Can you work these out from the model? Positions are in its coordinate system, mm. A direction names the side the tool comes from. Give positions to 0.01 mm unless a question says otherwise; leave off trailing zeros. Loops run counter-clockwise (first coordinate to the right, second up) from the corner with the lowest first, then second, coordinate; pieces in that order, holes last. Notation, with made-up numbers: (53.5, -12.5) - (95.5, -12.5) arc R23 ccw to (95.5, -4.5) - close; hole circle Ø6 at (4.25, 79). An arc over 180 degrees is marked (long way). Write item = value, one per line.
from build123d import *

# Parameters (mm, degrees)
SKETCH1_W           = 70
SKETCH1_H           = 100
BOSS_EXTRUDE1_DEPTH = 30
SKETCH2_R           = 4
BOSS_EXTRUDE2_DEPTH = 4
SKETCH3_W           = 35
SKETCH3_H           = 100
BOSS_EXTRUDE3_DEPTH = 40
SKETCH4_R           = 10
BOSS_EXTRUDE4_DEPTH = 17.5
BOSS_EXTRUDE5_DEPTH = 10
SKETCH6_W           = 150
SKETCH6_H           = 189.781220368
BOSS_EXTRUDE6_DEPTH = 10
SKETCH7_W           = 40
SKETCH7_H           = 189.781220368
BOSS_EXTRUDE7_DEPTH = 75


with BuildPart() as part:
    # Sketch1 → Boss-Extrude1 (new body)
    with BuildSketch(Plane(origin=(0, 0, 0), x_dir=(1, 0, 0), z_dir=(0, 1, 0))):
        Rectangle(SKETCH1_W, SKETCH1_H)
    extrude(amount=BOSS_EXTRUDE1_DEPTH)

    # Sketch2 → Boss-Extrude2 (add)
    # profile 1 of 4: a face of its own
    with BuildSketch(Plane(origin=(0, 30, 0), x_dir=(1, 0, 0), z_dir=(0, 1, 0))):
        with Locations(Location((-20, -35, 0), (0, 0, 270))):
            Circle(SKETCH2_R)
        Polygon((-18.132531053, -36.656757487), (-17.631471454, -34.211103194), (-19.498940402, -32.554345707), (-21.867468947, -33.343242513), (-22.368528546, -35.788896806), (-20.501059598, -37.445654293), align=None, mode=Mode.SUBTRACT)
    # profile 2 of 4: a face of its own
    with BuildSketch(Plane(origin=(0, 30, 0), x_dir=(1, 0, 0), z_dir=(0, 1, 0))):
        with Locations(Location((20, -35, 0), (0, 0, 270))):
            Circle(SKETCH2_R)
        Polygon((21.913058762, -37.035169602), (22.719037957, -34.360827314), (20.805979195, -32.325657712), (18.086941238, -32.964830398), (17.280962043, -35.639172686), (19.194020805, -37.674342288), align=None, mode=Mode.SUBTRACT)
    # profile 3 of 4: a face of its own
    with BuildSketch(Plane(origin=(0, 30, 0), x_dir=(1, 0, 0), z_dir=(0, 1, 0))):
        with Locations(Location((20, 0, 0), (0, 0, 270))):
            Circle(SKETCH2_R)
        Polygon((21.913058762, -1.47020522), (22.229764451, 0.921654877), (20.316705689, 2.391860097), (18.086941238, 1.47020522), (17.770235549, -0.921654877), (19.683294311, -2.391860097), align=None, mode=Mode.SUBTRACT)
    # profile 4 of 4: a face of its own
    with BuildSketch(Plane(origin=(0, 30, 0), x_dir=(1, 0, 0), z_dir=(0, 1, 0))):
        with Locations(Location((20, 35, 0), (0, 0, 270))):
            Circle(SKETCH2_R)
        Polygon((21.913058762, 33.534680981), (22.225532876, 35.924097978), (20.312474114, 37.389416996), (18.086941238, 36.465319019), (17.774467124, 34.075902022), (19.687525886, 32.610583004), align=None, mode=Mode.SUBTRACT)
    extrude(amount=BOSS_EXTRUDE2_DEPTH)

    # Sketch3 → Boss-Extrude3 (add)
    with BuildSketch(Plane.XZ):
        Rectangle(SKETCH3_W, SKETCH3_H)
    extrude(amount=BOSS_EXTRUDE3_DEPTH)

    # Sketch4 → Boss-Extrude4 (add)
    with BuildSketch(Plane(origin=(17.5, 0, 0), x_dir=(0, 0, -1), z_dir=(1, 0, 0))):
        with BuildLine():
            Line((-50, -40), (-139.781220368, -40))
            Line((-139.781220368, -40), (-129.48544067, 4.507505064))
            ThreePointArc((-129.48544067, 4.507505064), (-107.731609976, 19.87094378), (-90, 0))
            Line((-90, 0), (-50, 0))
            Line((-50, 0), (50, 0))
            Line((50, 0), (50, -40))
            Line((50, -40), (-50, -40))
        make_face()
        with Locations(Location((-110, 0, 0), (0, 0, 180))):
            Circle(SKETCH4_R, mode=Mode.SUBTRACT)
    extrude(amount=BOSS_EXTRUDE4_DEPTH)

    # Sketch5 → Boss-Extrude5 (add)
    with BuildSketch(Plane.XZ.offset(40)):
        Polygon((17.5, 139.781220368), (35, 139.781220368), (35, -50), (-17.5, -50), (-17.5, 50), (17.5, 50), align=None)
    extrude(amount=BOSS_EXTRUDE5_DEPTH)

    # Sketch6 → Boss-Extrude6 (add)
    with BuildSketch(Plane.XZ.offset(50)):
        with Locations((-40, 44.890610184)):
            Rectangle(SKETCH6_W, SKETCH6_H)
    extrude(amount=BOSS_EXTRUDE6_DEPTH)

    # Sketch7 → Boss-Extrude7 (add)
    with BuildSketch(Plane.XZ.offset(60)):
        with Locations((-40, 44.890610184)):
            Rectangle(SKETCH7_W, SKETCH7_H)
    extrude(amount=BOSS_EXTRUDE7_DEPTH)


solid = part.part
Q1. For pin 1 (1.3 mm diameter, centred on x = 19, z = -34.5, fed in from +Y); pin 2 (3 mm diameter, centred on x = 3, z = 83, fed in from -Y); pin 3 (2 mm diameter, centred on x = -86.5, z = -3.5, fed in from +Y); pin 4 (18 mm diameter, centred on y = 0, z = 110, fed in from +X), each with a flat end and sliding along its axis, tell me the tip position at first contact or that it passes through.
Output:
pin_1 = 30
pin_2 = -60
pin_3 = -50
pin_4 = through
Q2. Imagine slicing it at C-C, the plane x = 7. Write out the boundary of the cut face in (y, z).
Output:
outline = (-60, -50) - (30, -50) - (30, 50) - (-50, 50) - (-50, 139.78) - (-60, 139.78) - close
Q3. Which directions (+Z, -Z, +X, -X, +Y, -Y) give clear straight access to the entire face, cutting with the end or side of a thin tool? Please do faces 4 (the flat face through (-17.5, -25, -1)), 5 (the cylindrical face through (22.7, 31.97, -37.95)), 6 (the flat face through (-88, -60, 46)).
Output:
face_4 = +Z, -Z, -X
face_5 = +Y
face_6 = +Z, -Z, -X, -Y
Q4. I need wall thicknesses on L1, parallel to Y at x = -24, z = 20; L2, parallel to Y at x = -19, z = 22; L3, parallel to X at y = -122, z = 50. Which ranges of each line are inside material? Lowest first, please.
Output:
L1 = -135 to -50, 0 to 30
L2 = -60 to -50, 0 to 30
L3 = -60 to -20
Q5. Imagine slicing it at B-B, the plane z = 110. Write out the boundary of the cut face in (x, y).
Output:
outline = (-115, -60) - (-60, -60) - (-60, -135) - (-20, -135) - (-20, -60) - (35, -60) - (35, -10) - (17.5, -10) - (17.5, -50) - (-115, -50) - close; (17.5, 10) - (35, 10) - (35, 20) - (17.5, 20) - close
Q6. We'd pull the mould along X, two halves only. Please class faces 1 (the flat face through (-20, 30, 35)), 2 (the flat face through (17.5, -22, 94)), 3 (the flat face through (-40, -135, 46)): released by +X, released by -X, zero draft, split by the parting line, or undercut.
Output:
face_1 = undercut
face_2 = released by -X
face_3 = zero draft
Q7. Imagine slicing it at A-A, the plane z = 83. Write out the boundary of the cut face in (x, y).
Output:
outline = (-115, -60) - (-60, -60) - (-60, -135) - (-20, -135) - (-20, -60) - (35, -60) - (35, 0) - (17.5, 0) - (17.5, -50) - (-115, -50) - close
Q8. Imagine slicing it at D-D, the plane y = -44.5. Write out the boundary of the cut face in (x, z), then the cut area to 3 significant figures.
Output:
outline = (-17.5, -50) - (35, -50) - (35, 139.78) - (17.5, 139.78) - (17.5, 50) - (-17.5, 50) - close
area = 6,820 mm2
